Work out the finished part from the listing and answer in its coordinate system (mm). A direction names the side the tool comes from. Round coordinates to 2 decimals unless told otherwise and drop trailing zeros. Write each loop counter-clockwise with the first axis right and the second up, starting at its lowest first coordinate (ties: lowest second). Pieces come first, ordered by that corner, then holes. Notation, with made-up numbers: (-21, 40) -> (-12, 40) arc R20 cw to (-12, 67) -> close; hole circle Ø5 at (-37.5, 10). An arc over 180 degrees is marked (long way). One line per item, written item: value.
```python
from build123d import *

# Parameters (mm, degrees)
SKETCH1_W             = 8
SKETCH1_H             = 54
BOSS_EXTRUDE1_DEPTH   = 2.5
CUT_EXTRUDE1_DEPTH    = 28.748873851
M3_TAPPED_HOLE1_D     = 2.5
M3_TAPPED_HOLE1_DEPTH = 8.5
M3_TAPPED_HOLE1_TIP   = 0.751075774
CUT_EXTRUDE2_DEPTH    = 28.748873851
CHAMFER1_SIZE         = 0.5


with BuildPart() as part:
    # Sketch1 → Boss-Extrude1 (new, symmetric)
    with BuildSketch(Plane.XY):
        Rectangle(SKETCH1_W, SKETCH1_H)
    extrude(amount=BOSS_EXTRUDE1_DEPTH, both=True)

    # Sketch2 → Cut-Extrude1 (cut, through all)
    with BuildSketch(Plane.XY.offset(2.5)):
        Polygon((4, 27), (-4, 27), (-4, 25.946780019), align=None)
    extrude(amount=-CUT_EXTRUDE1_DEPTH, mode=Mode.SUBTRACT)

    # M3 Tapped Hole1
    with Locations(Plane(origin=(-3.425908761, 26.022360565, 0), x_dir=(0.9914448613738103, 0.13052619222005266, 0), z_dir=(-0.13052619222005266, 0.9914448613738103, 0))):
        with Locations((3.455470793, 0)):
            Hole(M3_TAPPED_HOLE1_D / 2, depth=M3_TAPPED_HOLE1_DEPTH)
            with Locations((0, 0, -(M3_TAPPED_HOLE1_DEPTH + M3_TAPPED_HOLE1_TIP / 2))):  # 118° drill point
                Cone(0, M3_TAPPED_HOLE1_D / 2, M3_TAPPED_HOLE1_TIP, mode=Mode.SUBTRACT)

    # Sketch5 → Cut-Extrude2 (cut, through all)
    with BuildSketch(Plane.XY.offset(2.5)):
        with BuildLine():
            Line((-1.6, -22), (-1.6, -16))
            ThreePointArc((-1.6, -16), (0, -14.4), (1.6, -16))
            Line((1.6, -16), (1.6, -22))
            ThreePointArc((1.6, -22), (0, -23.6), (-1.6, -22))
        make_face()
    extrude(amount=-CUT_EXTRUDE2_DEPTH, mode=Mode.SUBTRACT)

    # Chamfer1
    chamfer1_edges = [part.edges().sort_by_distance(p)[0] for p in [
        (-4, -0.52660999, -2.5),
        (-4, -0.52660999, 2.5),
        (4, 0, 2.5),
        (4, 0, -2.5),
    ]]
    chamfer(chamfer1_edges, length=CHAMFER1_SIZE)


solid = part.part
```
(1) Find section A-A on y = -18. Give the vertices of the cut face in (x, z).
Reported:
outline: (-4, -2) -> (-3.5, -2.5) -> (-1.6, -2.5) -> (-1.6, 2.5) -> (-3.5, 2.5) -> (-4, 2) -> close; (1.6, -2.5) -> (3.5, -2.5) -> (4, -2) -> (4, 2) -> (3.5, 2.5) -> (1.6, 2.5) -> close
(2) A flat-ended cylindrical pin translates along its axis: pin 1 Ø1.5 at (x, z) = (-1, 1) entering from +Y. Find the tip coordinate at first contact, or state that the pin passes through.
Reported:
pin 1: stops at y = 26.44
(3) For a pull along Z with two mould halves and no side action, classify faces 3 (the face through (0, 0, 2.5)), 4 (the face through (1.306, 17.446, -0.183)), 5 (the face through (0, -14.4, 0)), 6 (the face through (0, 0, -2.5)) as pulls with the +Z half, pulls with the -Z half, needs draft (parallel to the pull), parting line crosses it, or undercut.
Reported:
face 3: pulls with the +Z half
face 4: undercut
face 5: needs draft
face 6: pulls with the -Z half
(4) Consider probe 1 along X at (y, z) = (-18, 2); probe 2 along X at (y, z) = (-23, -1.3); probe 3 along Y at (x, z) = (0.5, -1.5). Determine where each line is inside the solid, lowest interval first.
Reported:
probe 1: x = -4 to -1.6, 1.6 to 4
probe 2: x = -4 to -1.25, 1.25 to 4
probe 3: y = -27 to -23.52, -14.48 to 26.54
(5) Find section B-B on x = -3. Give the vertices of the cut face in (y, z).
Reported:
outline: (-27, -2.5) -> (26.08, -2.5) -> (26.08, 2.5) -> (-27, 2.5) -> close
(6) A tool of negligible diameter and unlimited length cuts with its end or side. For faces 1 (the face through (0, -27, 0)), 2 (the face through (0, -23.6, 0)), from which of +Z, -Z, +X, -X, +Y, -Y can it reach the whole face along a straight path? Write none if from no direction.
Reported:
face 1: +Z, -Z, +X, -X, -Y
face 2: +Z, -Z
